Here's how the part is built. I have some questions about the finished solid (model axes, mm). A direction names the side the tool comes from. Give positions to 0.01 mm unless a question says otherwise; leave off trailing zeros. Write each loop counter-clockwise with the first axis right and the second up, starting at its lowest first coordinate (ties: lowest second). Pieces come first, ordered by that corner, then holes. Notation, with made-up numbers: (-22.75, 37) -> (11.25, 37) arc R14 ccw to (11.25, 64) -> close; hole circle Ø1 at (-29.75, 67.25). An arc over 180 degrees is marked (long way). Use one line per item in the form item = value.
```python
from build123d import *

# Parameters (mm, degrees)
BASE_PLATE_8MM_DEPTH      = 8
UPRIGHT_LOWER_15MM_DEPTH  = 15
UPRIGHT_MIDDLE_15MM_DEPTH = 15
UPRIGHT_TOP_SKETCH_W      = 10
UPRIGHT_TOP_SKETCH_H      = 40
UPRIGHT_TOP_10MM_DEPTH    = 10
SLOPE_CUT_DEPTH           = 40
CENTRE_SLOT_CUT_DEPTH     = 40
FRONT_NOTCH_CUT_DEPTH     = 40


with BuildPart() as part:
    # Base Plate Sketch → Base Plate 8mm (new body)
    with BuildSketch(Plane(origin=(0, 0, 0), x_dir=(1, 0, 0), z_dir=(0, 1, 0))):
        Polygon((0, 0), (20, 0), (20, 60), (-20, 60), (-20, 0), align=None)
    extrude(amount=BASE_PLATE_8MM_DEPTH)

    # Upright Lower Sketch → Upright Lower 15mm (add)
    with BuildSketch(Plane(origin=(20, 0, 0), x_dir=(0, 0, -1), z_dir=(1, 0, 0))):
        Polygon((60, 8), (60, 30), (45, 30), (20, 8), align=None)
    extrude(amount=-UPRIGHT_LOWER_15MM_DEPTH)

    # Upright Middle Sketch → Upright Middle 15mm (add)
    with BuildSketch(Plane.ZY.offset(20)):
        Polygon((-60, 8), (-60, 30), (-45, 30), (-20, 8), align=None)
    extrude(amount=-UPRIGHT_MIDDLE_15MM_DEPTH)

    # Upright Top Sketch → Upright Top 10mm (add)
    with BuildSketch(Plane(origin=(0, 8, 0), x_dir=(1, 0, 0), z_dir=(0, 1, 0))):
        with Locations((0, 40)):
            Rectangle(UPRIGHT_TOP_SKETCH_W, UPRIGHT_TOP_SKETCH_H)
    extrude(amount=UPRIGHT_TOP_10MM_DEPTH)

    # Slope Cut Sketch → Slope Cut (cut)
    with BuildSketch(Plane(origin=(5, 0, 0), x_dir=(0, 0, -1), z_dir=(1, 0, 0))):
        Polygon((20, 8), (20, 18), (31.363636364, 18), align=None)
    extrude(amount=-SLOPE_CUT_DEPTH, mode=Mode.SUBTRACT)

    # Centre Slot Sketch → Centre Slot Cut (cut)
    with BuildSketch(Plane(origin=(0, 0, -60), x_dir=(-1, 0, 0), z_dir=(0, 0, -1))):
        Polygon((0, 13), (15, 13), (15, 18), (-15, 18), (-15, 13), align=None)
    extrude(amount=-CENTRE_SLOT_CUT_DEPTH, mode=Mode.SUBTRACT)

    # Front Notch Sketch → Front Notch Cut (cut)
    with BuildSketch(Plane(origin=(0, 8, 0), x_dir=(1, 0, 0), z_dir=(0, 1, 0))):
        Polygon((0, 5), (10, 5), (10, 0), (-10, 0), (-10, 5), align=None)
    extrude(amount=-FRONT_NOTCH_CUT_DEPTH, mode=Mode.SUBTRACT)


solid = part.part
```
Q1. I want a section at C-C, the plane z = -46. Write out the boundary of the cut face in (x, y).
Result set:
outline = (-20, 0) -> (20, 0) -> (20, 30) -> (5, 30) -> (5, 18) -> (15, 18) -> (15, 13) -> (-15, 13) -> (-15, 18) -> (-5, 18) -> (-5, 30) -> (-20, 30) -> close
Q2. I want a section at B-B, the plane y = 23.25. Write out the boundary of the cut face in (x, z).
Result set:
outline = (-20, -60) -> (-5, -60) -> (-5, -37.33) -> (-20, -37.33) -> close; (5, -60) -> (20, -60) -> (20, -37.33) -> (5, -37.33) -> close
Q3. I want a section at A-A, the plane x = -9. Write out the boundary of the cut face in (y, z).
Result set:
outline = (0, -60) -> (13, -60) -> (13, -25.68) -> (8, -20) -> (8, -5) -> (0, -5) -> close; (18, -60) -> (30, -60) -> (30, -45) -> (18, -31.36) -> close
Q4. If we mould it in two halves opening along X, with no side actions, what happens to faces 6 (the face through (20, 12, -36)), 7 (the face through (15, 16, -43)), 8 (the face through (0, 11, -60))? For each: +X half, -X half, draft (parallel to the pull), parting line (faces both ways), or undercut.
Result set:
face_6 = +X half
face_7 = undercut
face_8 = draft
Q5. I want a section at D-D, the plane y = 3. Write out the boundary of the cut face in (x, z).
Result set:
outline = (-20, -60) -> (20, -60) -> (20, 0) -> (10, 0) -> (10, -5) -> (-10, -5) -> (-10, 0) -> (-20, 0) -> close
Q6. Will these pins go through, and if not, where does the flat tip stop? pin 1 Ø4 at (x, y) = (3.5, 5) entering from +Z; pin 2 Ø22 at (x, z) = (2.5, -15) entering from +Y.
Result set:
pin_1 = -5
pin_2 = 13
Q7. If I drill on line 1 along X through (y, z) = (27, -55); line 2 along X through (y, z) = (15.25, -44); line 3 along Y through (x, z) = (-7, -49.5), over which ranges is the centre line in solid material (lowest first)? Write a range as from..to.
Result set:
line_1 = -20..-5, 5..20
line_2 = -20..-15, 15..20
line_3 = 0..13, 18..30
Q8. Which directions (+Z, -Z, +X, -X, +Y, -Y) give clear straight access to the entire face, cutting with the end or side of a thin tool? Please do faces 1 (the face through (0, 13, -43)), 2 (the face through (0, 8, -10)), 3 (the face through (-13, 30, -53)), 4 (the face through (-5, 24, -49)), 5 (the face through (-10, 4, -2)).
Result set:
face_1 = +Z, -Z
face_2 = +Z, +X, -X, +Y
face_3 = +Z, -Z, +X, -X, +Y
face_4 = +Z, -Z, +Y
face_5 = +Z, +Y, -Y
